```python
from build123d import *

# Parameters (mm, degrees)
SKETCH_1_W                = 180
SKETCH_1_H                = 30
EXTRUDE_1_DEPTH           = 20
SKETCH_4_W                = 30
SKETCH_4_H                = 15
EXTRUDE_2_DEPTH           = 20
FILLET_1_R                = 5
CHAMFER_1_SIZE            = 5
HOLE_WIZARD_M8_2_D        = 6.8
HOLE_WIZARD_M8_2_DEPTH    = 19.75
HOLE_WIZARD_M8_2_TIP      = 2.042926105
HOLE_WIZARD_1_D           = 9
HOLE_WIZARD_1_DEPTH       = 27.5
HOLE_WIZARD_1_CBORE_D     = 15
HOLE_WIZARD_1_CBORE_DEPTH = 9
HOLE_WIZARD_1_TIP         = 2.703872786


with BuildPart() as part:
    # 草图1 → 凸台-拉伸1 (new body)
    with BuildSketch(Plane.XY):
        Rectangle(SKETCH_1_W, SKETCH_1_H)
    extrude(amount=EXTRUDE_1_DEPTH)

    # 草图4 → 凸台-拉伸2 (add)
    with BuildSketch(Plane.XY.offset(20)):
        with Locations((75, -22.5)):
            Rectangle(SKETCH_4_W, SKETCH_4_H)
    extrude(amount=-EXTRUDE_2_DEPTH)

    # 圆角1
    fillet_1_edges = [part.edges().sort_by_distance(p)[0] for p in [
        (60, -15, 10),
    ]]
    fillet(fillet_1_edges, radius=FILLET_1_R)

    # 倒角1
    chamfer_1_edges = [part.edges().sort_by_distance(p)[0] for p in [
        (90, 15, 10),
    ]]
    chamfer(chamfer_1_edges, length=CHAMFER_1_SIZE)

    # M8 螺纹孔2
    with Locations(Plane(origin=(0, -30, 0), x_dir=(-1, 0, 0), z_dir=(0, -1, 0))):
        with Locations((-75, -10)):
            Hole(HOLE_WIZARD_M8_2_D / 2, depth=HOLE_WIZARD_M8_2_DEPTH)
            with Locations((0, 0, -(HOLE_WIZARD_M8_2_DEPTH + HOLE_WIZARD_M8_2_TIP / 2))):  # 118° drill point
                Cone(0, HOLE_WIZARD_M8_2_D / 2, HOLE_WIZARD_M8_2_TIP, mode=Mode.SUBTRACT)

    # 打孔尺寸(%根据)内六角圆柱头螺钉的类型1
    with Locations(Plane(origin=(0, 0, 0), x_dir=(-1, 0, 0), z_dir=(0, 0, -1))):
        with Locations((65, 0), (5, 0)):
            CounterBoreHole(HOLE_WIZARD_1_D / 2, HOLE_WIZARD_1_CBORE_D / 2, HOLE_WIZARD_1_CBORE_DEPTH, depth=HOLE_WIZARD_1_DEPTH)
            with Locations((0, 0, -(HOLE_WIZARD_1_DEPTH + HOLE_WIZARD_1_TIP / 2))):  # 118° drill point
                Cone(0, HOLE_WIZARD_1_D / 2, HOLE_WIZARD_1_TIP, mode=Mode.SUBTRACT)


solid = part.part
```
Geometry: final body of the model. Coordinates: model frame, mm. A direction names the side the tool comes from. Give positions to 0.01 mm unless a question says otherwise; leave off trailing zeros. Loops run counter-clockwise (first coordinate to the right, second up) from the corner with the lowest first, then second, coordinate; pieces in that order, holes last. Notation, with made-up numbers: (-18.75, -21) -> (33.25, -21) arc R25 cw to (33.25, 3) -> close; hole circle Ø4 at (81, 47.25). An arc over 180 degrees is marked (long way). Return JSON: item names as keys, results as strings.
Item 1: Pin query (flat end, axial travel): P1, Ø12, axis at x = -68.5, z = 8.5, coming from the -Y side; P2, Ø5, axis at y = -25, z = 10.5, coming from the -X side; P3, Ø4.5, axis at x = -61.5, y = -2.5, coming from the -Z side. Return the tip coordinate at first contact, or that it passes through.
Filled in:
{"P1": "y = -15", "P2": "x = 60", "P3": "z = 9"}
Item 2: Line query: line 1 (X direction, y = -6, z = 3); line 2 (Y direction, x = -5, z = 7); line 3 (X direction, y = 1, z = 10). Output: solid intervals per line, ascending.
Filled in:
{"line 1": "-90 to -69.5, -60.5 to -9.5, -0.5 to 90", "line 2": "-15 to -7.5, 7.5 to 15", "line 3": "-90 to -69.39, -60.61 to -9.39, -0.61 to 90"}
Item 3: Section B-B, the plane x = -65. Output: boundary loops of the cut face in (y, z), plus the area to 3 significant figures.
Filled in:
{"outline": "(-15, 0) -> (-7.5, 0) -> (-7.5, 9) -> (-4.5, 9) -> (-4.5, 20) -> (-15, 20) -> close; (4.5, 9) -> (7.5, 9) -> (7.5, 0) -> (15, 0) -> (15, 20) -> (4.5, 20) -> close", "area": "366 mm^2"}
Item 4: Section C-C, the plane z = 18. Output: boundary loops of the cut face in (x, y), plus the area to 3 significant figures.
Filled in:
{"outline": "(-90, -15) -> (55, -15) arc R5 cw to (60, -20) -> (60, -30) -> (90, -30) -> (90, 10) -> (85, 15) -> (-90, 15) -> close; hole circle Ø9 at (-65, 0); hole circle Ø9 at (-5, 0)", "area": "5,720 mm^2"}
Item 5: Access query for faces 1 (the flat face through (-19, -15, 10)), 2 (the flat face through (-10, 0, 9)), 3 (the flat face through (-4, 15, 10)). Directions: +Z, -Z, +X, -X, +Y, -Y. A direction counts if a zero-diameter tool reaches every point of the face in a straight line with its end or side. Return the directions, or none.
Filled in:
{"face 1": "+Z, -Z, -X, -Y", "face 2": "-Z", "face 3": "+Z, -Z, +X, -X, +Y"}
Item 6: Section A-A, the plane y = 0. Output: boundary loops of the cut face in (x, z), plus the area to 3 significant figures.
Filled in:
{"outline": "(-90, 0) -> (-72.5, 0) -> (-72.5, 9) -> (-69.5, 9) -> (-69.5, 20) -> (-90, 20) -> close; (-60.5, 9) -> (-57.5, 9) -> (-57.5, 0) -> (-12.5, 0) -> (-12.5, 9) -> (-9.5, 9) -> (-9.5, 20) -> (-60.5, 20) -> close; (-0.5, 9) -> (2.5, 9) -> (2.5, 0) -> (90, 0) -> (90, 20) -> (-0.5, 20) -> close", "area": "3,130 mm^2"}
Item 7: Mould query, pull axis Z, two halves, no side actions, for faces 4 (the cylindrical face through (72.302, -19.987, 12.069)), 5 (the flat face through (-65, -5, 9)), 6 (the flat face through (60, -25, 10)). Classes: released by +Z, released by -Z, zero draft, split by the parting line, or undercut.
Filled in:
{"face 4": "undercut", "face 5": "released by -Z", "face 6": "zero draft"}
Item 8: Section D-D, the plane z = 2. Output: boundary loops of the cut face in (x, y), plus the area to 3 significant figures.
Filled in:
{"outline": "(-90, -15) -> (55, -15) arc R5 cw to (60, -20) -> (60, -30) -> (90, -30) -> (90, 10) -> (85, 15) -> (-90, 15) -> close; hole circle Ø15 at (-65, 0); hole circle Ø15 at (-5, 0)", "area": "5,490 mm^2"}
